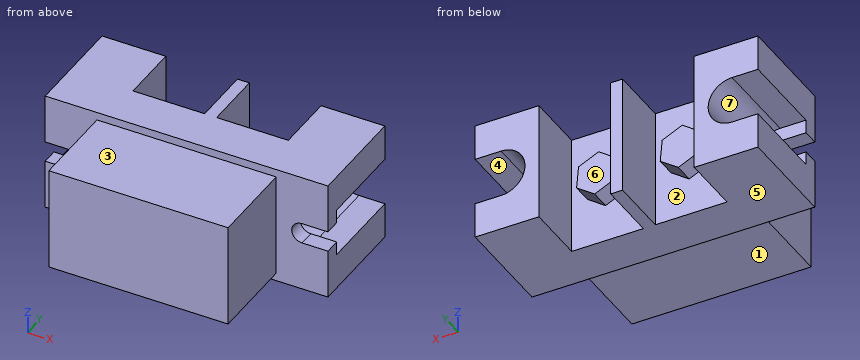
from build123d import *

# Parameters (mm, degrees)
SKETCH_1_W             = 71
SKETCH_1_H             = 30
EXTRUDE_1_DEPTH        = 26
SKETCH_2_W             = 45
SKETCH_2_H             = 26
EXTRUDE_2_DEPTH        = 22
CUT_EXTRUDE_1_DEPTH    = 62.556884262
CUT_EXTRUDE_2_DEPTH    = 22
SKETCH_5_W             = 18
SKETCH_5_H             = 30
CUT_EXTRUDE_3_DEPTH    = 15
PATTERN_LINEAR_1_COUNT = 2
PATTERN_LINEAR_1_PITCH = 21
EXTRUDE_3_DEPTH        = 5
PATTERN_LINEAR_2_COUNT = 2
PATTERN_LINEAR_2_PITCH = 21


with BuildPart() as part:
    # 草图1 → 凸台-拉伸1 (new body)
    with BuildSketch(Plane(origin=(0, 0, 0), x_dir=(1, 0, 0), z_dir=(0, 1, 0))):
        Rectangle(SKETCH_1_W, SKETCH_1_H)
    extrude(amount=EXTRUDE_1_DEPTH)

    # 草图2 → 凸台-拉伸2 (add)
    with BuildSketch(Plane.XZ):
        Rectangle(SKETCH_2_W, SKETCH_2_H)
    extrude(amount=EXTRUDE_2_DEPTH)

    # 草图3 → 切除-拉伸1 (cut, through all)
    with BuildSketch(Plane(origin=(0, 26, 0), x_dir=(1, 0, 0), z_dir=(0, 1, 0))):
        with BuildLine():
            Line((-29, -2.6), (-61.70015948, -2.6))
            ThreePointArc((-61.70015948, -2.6), (-64.30015948, 0), (-61.70015948, 2.6))
            Line((-61.70015948, 2.6), (-29, 2.6))
            ThreePointArc((-29, 2.6), (-26.4, 0), (-29, -2.6))
        make_face()
        with BuildLine():
            Line((29, 2.6), (61.70015948, 2.6))
            ThreePointArc((61.70015948, 2.6), (64.30015948, 0), (61.70015948, -2.6))
            Line((61.70015948, -2.6), (29, -2.6))
            ThreePointArc((29, -2.6), (26.4, 0), (29, 2.6))
        make_face()
    extrude(amount=-CUT_EXTRUDE_1_DEPTH, mode=Mode.SUBTRACT)

    # 草图4 → 切除-拉伸2 (cut)
    with BuildSketch(Plane(origin=(0, 26, 0), x_dir=(1, 0, 0), z_dir=(0, 1, 0))):
        with BuildLine():
            Line((29, 6), (52.513840992, 6))
            ThreePointArc((52.513840992, 6), (58.513840992, 0), (52.513840992, -6))
            Line((52.513840992, -6), (29, -6))
            ThreePointArc((29, -6), (23, 0), (29, 6))
        make_face()
        with BuildLine():
            Line((-29, -6), (-53.007180335, -6))
            ThreePointArc((-53.007180335, -6), (-59.007180335, 0), (-53.007180335, 6))
            Line((-53.007180335, 6), (-29, 6))
            ThreePointArc((-29, 6), (-23, 0), (-29, -6))
        make_face()
    extrude(amount=-CUT_EXTRUDE_2_DEPTH, mode=Mode.SUBTRACT)

    # 草图5 → 切除-拉伸3 (cut)
    with BuildSketch(Plane(origin=(0, 26, 0), x_dir=(1, 0, 0), z_dir=(0, 1, 0))):
        with Locations((10.5, 0)):
            Rectangle(SKETCH_5_W, SKETCH_5_H)
    cut_extrude_3 = extrude(amount=-CUT_EXTRUDE_3_DEPTH, mode=Mode.SUBTRACT)

    # 阵列(线性)1: 切除-拉伸3 ×2
    with Locations(*[(-i * PATTERN_LINEAR_1_PITCH, 0, 0) for i in range(1, PATTERN_LINEAR_1_COUNT)]):
        add(cut_extrude_3, mode=Mode.SUBTRACT)

    # 草图6 → 凸台-拉伸3 (add)
    with BuildSketch(Plane(origin=(0, 11, 0), x_dir=(1, 0, 0), z_dir=(0, 1, 0))):
        Polygon((15.033036482, -3.195715708), (15.534089227, 2.327866896), (11.001052745, 5.523582603), (5.966963518, 3.195715708), (5.465910773, -2.327866896), (9.998947255, -5.523582603), align=None)
    extrude_3 = extrude(amount=EXTRUDE_3_DEPTH)

    # 阵列(线性)2: 凸台-拉伸3 ×2
    with Locations(*[(-i * PATTERN_LINEAR_2_PITCH, 0, 0) for i in range(1, PATTERN_LINEAR_2_COUNT)]):
        add(extrude_3)


solid = part.part
Geometry check sheet. Reference: the model listing, model coordinates, mm. Face numbers are marked on the shaded views. A direction names the side the tool comes from. Round coordinates to 2 decimals unless told otherwise and drop trailing zeros. Write each loop counter-clockwise with the first axis right and the second up, starting at its lowest first coordinate (ties: lowest second). Pieces come first, ordered by that corner, then holes.
Item 1: Material ranges on line 1 along X through (y, z) = (17.5, -12.5); line 2 along Y through (x, z) = (12, -4); line 3 along Y through (x, z) = (25, -2), recorded low to high.
Determined:
line 1: x = -35.5 to -19.5, -1.5 to 1.5, 19.5 to 35.5
line 2: y = -22 to 16
line 3: y = 0 to 4
Item 2: Mould release check, pull along Z, two halves, no side actions. Record for the marked faces 5, 6 and 7: +Z half, -Z half, draft (parallel to the pull), parting line (faces both ways), or undercut.
Determined:
face 5: -Z half
face 6: draft
face 7: undercut
Item 3: Section check D-D (y = -3). Record the boundary of the cut face in (x, z), plus the area to 3 significant figures.
Determined:
outline: (-22.5, -13) - (22.5, -13) - (22.5, 13) - (-22.5, 13) - close
area: 1,170 mm2
Item 4: Access from +Z, -Z, +X, -X, +Y, -Y to the whole of each face (thin tool, end or side, straight path). Record for the marked faces 1, 2, 3 and 4.
Determined:
face 1: -Z, +X, -X, -Y
face 2: +Y
face 3: +Z, +X, -X, -Y
face 4: +X, +Y
Item 5: Go/stop test with flat-tipped pins: pin 1 Ø1.5 at (x, z) = (28, -6.5) entering from -Y; pin 2 Ø17.5 at (y, z) = (-14, -3.5) entering from +X; pin 3 Ø1 at (x, y) = (-19, -6) entering from -Z. Record where each tip stops, or that it passes through.
Determined:
pin 1: stops at y = 0
pin 2: stops at x = 22.5
pin 3: stops at z = -13
Item 6: Section check A-A (y = 17). Record the boundary of the cut face in (x, z), plus the area to 3 significant figures.
Determined:
outline: (-35.5, -15) - (-19.5, -15) - (-19.5, 15) - (-35.5, 15) - (-35.5, 6) - (-29, 6) arc R6 cw to (-29, -6) - (-35.5, -6) - close; (-1.5, -15) - (1.5, -15) - (1.5, 15) - (-1.5, 15) - close; (19.5, -15) - (35.5, -15) - (35.5, -6) - (29, -6) arc R6 cw to (29, 6) - (35.5, 6) - (35.5, 15) - (19.5, 15) - close
area: 781 mm2
Item 7: Section check B-B (z = -10). Record the boundary of the cut face in (x, y).
Determined:
outline: (-35.5, 0) - (-22.5, 0) - (-22.5, -22) - (22.5, -22) - (22.5, 0) - (35.5, 0) - (35.5, 26) - (19.5, 26) - (19.5, 11) - (1.5, 11) - (1.5, 26) - (-1.5, 26) - (-1.5, 11) - (-19.5, 11) - (-19.5, 26) - (-35.5, 26) - close
Item 8: Section check C-C (x = 18.5). Record the boundary of the cut face in (y, z).
Determined:
outline: (-22, -13) - (0, -13) - (0, -15) - (11, -15) - (11, 15) - (0, 15) - (0, 13) - (-22, 13) - close
